```python
from build123d import *

# Parameters (mm, degrees)
SKETCH_1_W                  = 153.5
SKETCH_1_H                  = 80
EXTRUDE_1_DEPTH             = 7.5
HOLE_WIZARD_25_0_25_1_D     = 25
HOLE_WIZARD_M8_1_AT_2_COUNT = 2
HOLE_WIZARD_M8_1_AT_2_PITCH = 60
CHAMFER_1_SIZE              = 2


with BuildPart() as part:
    # 草图1 → 凸台-拉伸1 (new, symmetric)
    with BuildSketch(Plane.XY):
        Rectangle(SKETCH_1_W, SKETCH_1_H)
    extrude(amount=EXTRUDE_1_DEPTH, both=True)

    # Ø25.0 (25) 直径孔1 (through all)
    with Locations(Plane.XY.offset(7.5)):
        with Locations((36.75, 0)):
            Hole(HOLE_WIZARD_25_0_25_1_D / 2)

    # 草图4 → M8 螺纹孔1 (revolve, cut)
    with BuildSketch(Plane(origin=(76.75, 30, 0), x_dir=(0, 0, -1), z_dir=(0, 1, 0))):
        Polygon((0, 0), (0, 21.792926105), (3.4, 19.75), (3.4, 0), align=None)
    hole_wizard_m8_1 = revolve(axis=Axis((83.1, 30, 0), (-1, 0, 0)), mode=Mode.SUBTRACT)

    # M8 螺纹孔1 at 2: M8 螺纹孔1 ×2
    with Locations(*[(0, -i * HOLE_WIZARD_M8_1_AT_2_PITCH, 0) for i in range(1, HOLE_WIZARD_M8_1_AT_2_COUNT)]):
        add(hole_wizard_m8_1, mode=Mode.SUBTRACT)

    # 镜向1: M8 螺纹孔1 across plane
    add(hole_wizard_m8_1.mirror(Plane(origin=(0, 0, 0), x_dir=(0, 0, 1), z_dir=(1, 0, 0))), mode=Mode.SUBTRACT)

    # 镜向1 copy 1 sketch → 镜向1 copy 1 (revolve, cut)
    with BuildSketch(Plane(origin=(-76.75, -30, 0), x_dir=(0, 0, -1), z_dir=(0, 1, 0))):
        Polygon((0, 0), (0, -21.792926105), (3.4, -19.75), (3.4, 0), align=None)
    revolve(axis=Axis((-83.1, -30, 0), (-1, 0, 0)), mode=Mode.SUBTRACT)

    # 倒角1
    chamfer_1_edges = [part.edges().sort_by_distance(p)[0] for p in [
        (76.75, -40, 0),
        (-76.75, -40, 0),
        (-76.75, 40, 0),
        (76.75, 40, 0),
    ]]
    chamfer(chamfer_1_edges, length=CHAMFER_1_SIZE)


solid = part.part
```
Model file for the job. Use its own axes, mm. A direction names the side the tool comes from. Give positions to 0.01 mm unless a question says otherwise; leave off trailing zeros. Loops run counter-clockwise (first coordinate to the right, second up) from the corner with the lowest first, then second, coordinate; pieces in that order, holes last. Notation, with made-up numbers: M 79,70 L 96,70 A23 cw 96,97 Z; hole C 63,56.5 d8. An arc over 180 degrees is marked long. Use one line per item in the form item = value.
Item 1: Which spindle directions (+Z, -Z, +X, -X, +Y, -Y) get a long thin tool onto all of the face, cutting with end or side? Do faces 1 (the flat face through (-1, -40, 0)), 2 (the cylindrical face through (-67.01, 26.63, 0.44)), 3 (the cylindrical face through (67.01, -26.68, 0.74)). Say none if no direction does.
Filled in:
face_1 = +Z, -Z, +X, -X, -Y
face_2 = -X
face_3 = +X
Item 2: Flat gauge pins, fed straight in: pin 1 Ø9 at (y, z) = (-30, 0) entering from +X; pin 2 Ø5.5 at (y, z) = (30, 0) entering from -X. Where does each tip first touch, or does it go through?
Filled in:
pin_1 = 76.75
pin_2 = -56.61
Item 3: Slice it at B-B on z = 6. List the corners of the cut face in (x, y).
Filled in:
outline = M -76.75,-38 L -74.75,-40 L 74.75,-40 L 76.75,-38 L 76.75,38 L 74.75,40 L -74.75,40 L -76.75,38 Z; hole C 36.75,0 d25
Item 4: Slice it at C-C on y = -8. List the corners of the cut face in (x, z), and give its area (3 significant figures).
Filled in:
outline = M -76.75,-7.5 L 27.15,-7.5 L 27.15,7.5 L -76.75,7.5 Z; M 46.35,-7.5 L 76.75,-7.5 L 76.75,7.5 L 46.35,7.5 Z
area = 2,010 mm^2
Item 5: Slice it at A-A on y = 10. List the corners of the cut face in (x, z), and give its area (3 significant figures).
Filled in:
outline = M -76.75,-7.5 L 29.25,-7.5 L 29.25,7.5 L -76.75,7.5 Z; M 44.25,-7.5 L 76.75,-7.5 L 76.75,7.5 L 44.25,7.5 Z
area = 2,080 mm^2
Item 6: Two-plate mould, pull along X, no slides. Class faces 4 (the conical face through (55.312, -29.424, 0.128)), 5 (the flat face through (-1, 1, 7.5)), 6 (the conical face through (-55.312, -29.424, 0.128)), 7 (the cylindrical face through (46.67, -7.606, -0.105)): released by +X, released by -X, zero draft, split by the parting line, or undercut.
Filled in:
face_4 = released by +X
face_5 = zero draft
face_6 = released by -X
face_7 = undercut
Item 7: Drill centre lines: L1, parallel to Y at x = 64, z = 0; L2, parallel to Z at x = -72.5, y = 30; L3, parallel to X at y = -4, z = 3.25. Where is each one in solid material? Low to high.
Filled in:
L1 = -40 to -33.4, -26.6 to 26.6, 33.4 to 40
L2 = -7.5 to -3.4, 3.4 to 7.5
L3 = -76.75 to 24.91, 48.59 to 76.75
